Part model, mm, in its own coordinate system. Face numbers are marked on the shaded views. A direction names the side the tool comes from. Coordinates: 2 decimals unless noted, no trailing zeros. Order: outer loops, then holes, each group sorted by start corner. A loop starts at its lowest first (then second) coordinate and runs counter-clockwise, first axis right, second up.
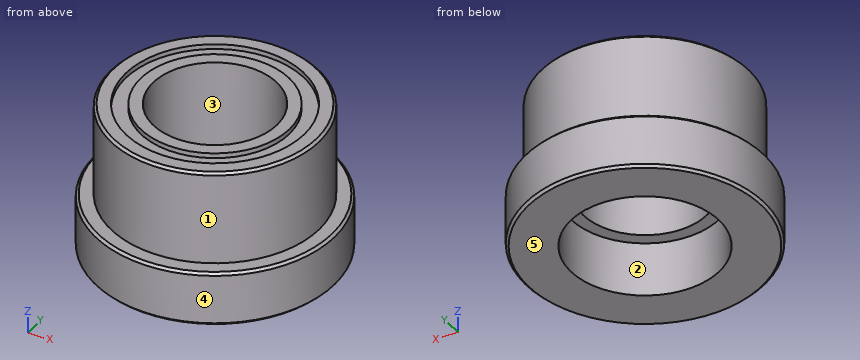
from build123d import *

# Parameters (mm, degrees)
SKETCH1_R           = 24.1
BOSS_EXTRUDE1_DEPTH = 11
SKETCH2_R           = 15
CUT_EXTRUDE1_DEPTH  = 36.813684535
SKETCH3_R           = 21
SKETCH3_R_2         = 12.5
BOSS_EXTRUDE2_DEPTH = 19
CHAMFER1_SIZE       = 0.5
SKETCH4_R           = 18
SKETCH4_R_2         = 15
CUT_EXTRUDE2_DEPTH  = 1


with BuildPart() as part:
    # Sketch1 → Boss-Extrude1 (new body)
    with BuildSketch(Plane.XY):
        Circle(SKETCH1_R)
    extrude(amount=BOSS_EXTRUDE1_DEPTH)

    # Sketch2 → Cut-Extrude1 (cut, through all)
    with BuildSketch(Plane.XY.offset(11)):
        Circle(SKETCH2_R)
    extrude(amount=-CUT_EXTRUDE1_DEPTH, mode=Mode.SUBTRACT)

    # Sketch3 → Boss-Extrude2 (add)
    with BuildSketch(Plane.XY.offset(11)):
        Circle(SKETCH3_R)
        Circle(SKETCH3_R_2, mode=Mode.SUBTRACT)
    extrude(amount=BOSS_EXTRUDE2_DEPTH)

    # Chamfer1
    chamfer1_edges = [part.edges().sort_by_distance(p)[0] for p in [
        (-21, 0, 30),
        (-24.1, 0, 0),
        (-24.1, 0, 11),
    ]]
    chamfer(chamfer1_edges, length=CHAMFER1_SIZE)

    # Sketch4 → Cut-Extrude2 (cut)
    with BuildSketch(Plane.XY.offset(30)):
        Circle(SKETCH4_R)
        Circle(SKETCH4_R_2, mode=Mode.SUBTRACT)
    extrude(amount=-CUT_EXTRUDE2_DEPTH, mode=Mode.SUBTRACT)


solid = part.part
Q1. Cut at D-D on z = 8.5. Write the cut outline in (x, y), and give its area (3 significant figures).
Results list:
outline: circle Ø48.2 at (0, 0); hole circle Ø30 at (0, 0)
area: 1,120 mm2
Q2. Cut at C-C on z = 19. Write the cut outline in (x, y), and give its area (3 significant figures).
Results list:
outline: circle Ø42 at (0, 0); hole circle Ø25 at (0, 0)
area: 895 mm2
Q3. Which spindle directions (+Z, -Z, +X, -X, +Y, -Y) get a long thin tool onto all of the face, cutting with end or side? Do the marked faces 1 and 2. Say none if no direction does.
Results list:
face 1: +Z
face 2: -Z
Q4. Pin check, flat tips, straight feed: pin 1 Ø10 at (x, z) = (-14, 22.5) entering from +Y; pin 2 Ø6 at (x, y) = (15, -17.5) entering from -Z; pin 3 Ø3 at (y, z) = (5, 23) entering from -X; pin 4 Ø6 at (x, z) = (-4.5, 6) entering from -Y. Stop position of each tip, or through.
Results list:
pin 1: stops at y = 18.97
pin 2: stops at z = 0
pin 3: stops at x = -20.71
pin 4: stops at y = -24.05
Q5. Mould opens along X. For the marked faces 3, 4 and 5 say: pulls with the +X half, pulls with the -X half, needs draft (parallel to the pull), parting line crosses it, or undercut.
Results list:
face 3: undercut
face 4: parting line crosses it
face 5: needs draft
Q6. Wall check: line 1 along Y through (x, z) = (0, 4); line 2 along Y through (x, z) = (0, 23.75); line 3 along Z through (x, y) = (-19.5, -12.5). Give the ranges that are in metal, low to high.
Results list:
line 1: y = -24.1 to -15, 15 to 24.1
line 2: y = -21 to -12.5, 12.5 to 21
line 3: z = 0 to 11
